from build123d import *

# Parameters (mm, degrees)
SKETCH1_W           = 200
SKETCH1_H           = 160
BOSS_EXTRUDE1_DEPTH = 6
FILLET1_R           = 6
M10_TAPPED_HOLE1_D  = 8.5


with BuildPart() as part:
    # Sketch1 → Boss-Extrude1 (new body)
    with BuildSketch(Plane(origin=(0, 0, 0), x_dir=(1, 0, 0), z_dir=(0, 1, 0))):
        Rectangle(SKETCH1_W, SKETCH1_H)
    extrude(amount=BOSS_EXTRUDE1_DEPTH)

    # Fillet1
    fillet1_edges = [part.edges().sort_by_distance(p)[0] for p in [
        (100, 3, 80),
        (-100, 3, 80),
        (-100, 3, -80),
        (100, 3, -80),
    ]]
    fillet(fillet1_edges, radius=FILLET1_R)

    # M10 Tapped Hole1 (through all)
    with Locations(Plane(origin=(0, 6, 0), x_dir=(1, 0, 0), z_dir=(0, 1, 0))):
        with Locations((0, 0), (42.5, 69), (-42.5, 69), (-89, 0), (89, 0), (42.5, -69), (-42.5, -69)):
            Hole(M10_TAPPED_HOLE1_D / 2)


solid = part.part
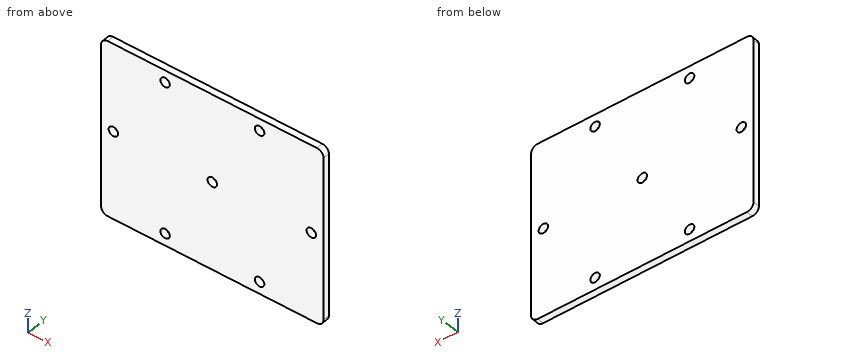
The listing builds one solid part. Answer for the finished solid, in the listing's coordinates (mm). Round coordinates to 2 decimals unless told otherwise and drop trailing zeros. Order: outer loops, then holes, each group sorted by start corner. A loop starts at its lowest first (then second) coordinate and runs counter-clockwise, first axis right, second up. Notation, with made-up numbers: (9.25, 1) - (51.25, 1) arc R23 ccw to (51.25, 22) - close; hole circle Ø11 at (9, 22). An arc over 180 degrees is marked (long way). Write item = value, one per line. Start each with the question number.
1) Straight lines are drawn through the part: L1, parallel to Z at x = 42.5, y = 4.6; L2, parallel to X at y = 3.6, z = 68.5; L3, parallel to Z at x = -40.5, y = 1. For each, find the intervals that lie inside material, in ascending order.
2) Given pin 1 (10 mm diameter, centred on x = -42.5, z = -69, fed in from +Y); pin 2 (7.5 mm diameter, centred on x = -42.5, z = 69, fed in from +Y), each flat-ended and moving along its own axis, determine where each tip first touches the part or whether it passes through.
3) Section C-C, the plane x = -89 is taken. Write down the section's boundary in (y, z).
4) Section A-A, the plane x = -42.5 is taken. Write down the section's boundary in (y, z).
5) Section D-D, the plane x = 1 is taken. Write down the section's boundary in (y, z), plus the area to 3 significant figures.
6) Section B-B, the plane z = 69 is taken. Write down the section's boundary in (x, y).
Results list:
q1.L1 = -80 to -73.25, -64.75 to 64.75, 73.25 to 80
q1.L2 = -100 to -46.72, -38.28 to 38.28, 46.72 to 100
q1.L3 = -80 to -72.75, -65.25 to 65.25, 72.75 to 80
q2.pin_1 = 6
q2.pin_2 = through
q3.outline = (0, -80) - (6, -80) - (6, -4.25) - (0, -4.25) - close; (0, 4.25) - (6, 4.25) - (6, 80) - (0, 80) - close
q4.outline = (0, -80) - (6, -80) - (6, -73.25) - (0, -73.25) - close; (0, -64.75) - (6, -64.75) - (6, 64.75) - (0, 64.75) - close; (0, 73.25) - (6, 73.25) - (6, 80) - (0, 80) - close
q5.outline = (0, -80) - (6, -80) - (6, -4.13) - (0, -4.13) - close; (0, 4.13) - (6, 4.13) - (6, 80) - (0, 80) - close
q5.area = 910 mm^2
q6.outline = (-100, 0) - (-46.75, 0) - (-46.75, 6) - (-100, 6) - close; (-38.25, 0) - (38.25, 0) - (38.25, 6) - (-38.25, 6) - close; (46.75, 0) - (100, 0) - (100, 6) - (46.75, 6) - close
